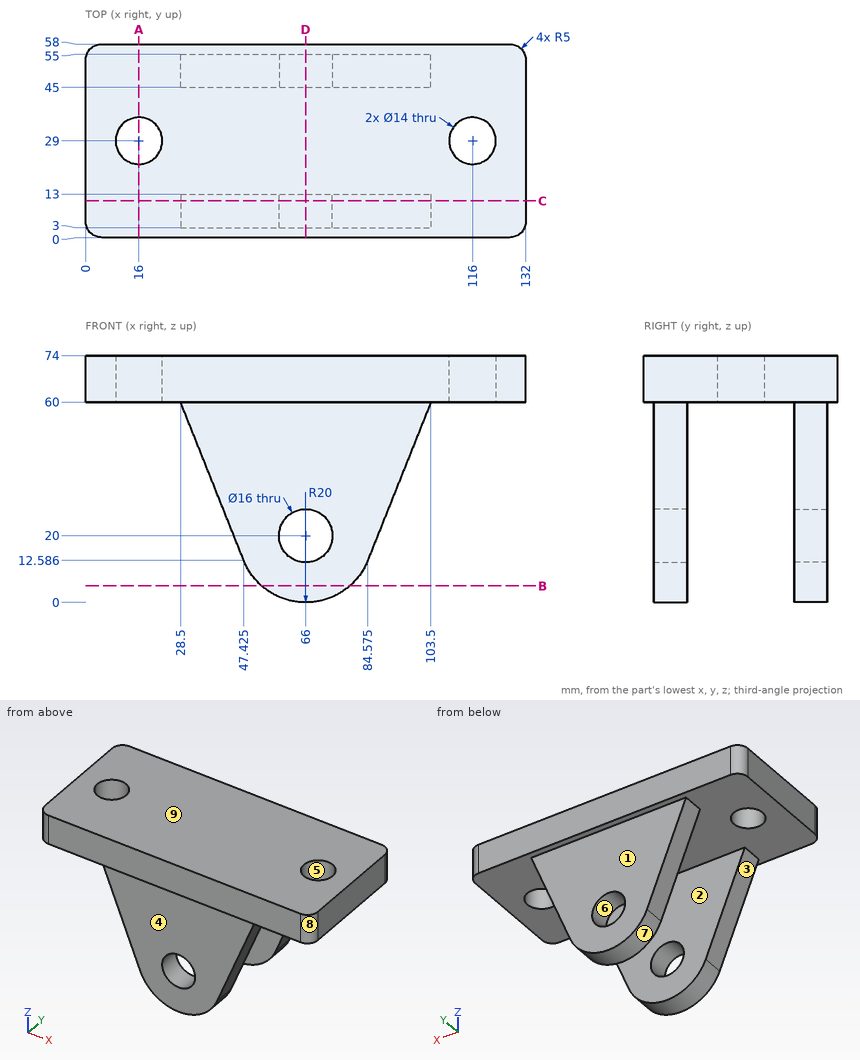
The figure shows three views and two pictorial views of one solid part (mm, origin at its lowest corner). Answer the questions. A direction names the side the tool comes from. Round coordinates to 2 decimals unless told otherwise and drop trailing zeros. Write each loop counter-clockwise with the first axis right and the second up, starting at its lowest first coordinate (ties: lowest second). Pieces come first, ordered by that corner, then holes. Notation, with made-up numbers: (25, 55) -> (51, 55) arc R21 ccw to (51, 76) -> close; hole circle Ø1 at (-25, 52.25). An arc over 180 degrees is marked (long way). Write each question's results on one line, items separated by ' | '.
Q1. Which of the six approach directions +Z, -Z, +X, -X, +Y, -Y give full straight-line access (tool end or side, diameter ignored) to the marked faces 1, 2, 3, 4 and 5?
Data:
face 1: -Z, +X, -X, +Y | face 2: -Z, +X, -X | face 3: -Z, -X, +Y, -Y | face 4: -Z, +X, -X, -Y | face 5: +Z, -Z
Q2. Section B-B, the plane z = 5 is taken. Write down the section's boundary in (x, y).
Data:
outline: (52.77, 3) -> (79.23, 3) -> (79.23, 13) -> (52.77, 13) -> close; (52.77, 45) -> (79.23, 45) -> (79.23, 55) -> (52.77, 55) -> close
Q3. Determine the mould class of the marked faces 6, 7, 8 and 9 for opening direction Z: released by +Z, released by -Z, zero draft, split by the parting line, or undercut.
Data:
face 6: undercut | face 7: released by -Z | face 8: zero draft | face 9: released by +Z
Q4. Flat-ended cylindrical pins translate along their axes: P1, Ø21, axis at x = 66, z = 20, coming from the -Y side; P2, Ø5, axis at y = 11, z = 17, coming from the -X side; P3, Ø18, axis at x = 60, z = 23, coming from the +Y side. Find the tip coordinate at first contact, or state that the pin passes through.
Data:
P1: y = 3 | P2: x = 44.67 | P3: y = 55
Q5. Section A-A, the plane x = 16 is taken. Write down the section's boundary in (y, z), then the cut area to 3 significant figures.
Data:
outline: (0, 60) -> (22, 60) -> (22, 74) -> (0, 74) -> close; (36, 60) -> (58, 60) -> (58, 74) -> (36, 74) -> close | area: 616 mm^2
Q6. Section C-C, the plane y = 11 is taken. Write down the section's boundary in (x, z) (3 decimals), then the cut area to 3 significant figures.
Data:
outline: (0, 60) -> (28.5, 60) -> (47.425, 12.586) arc R20 ccw to (84.575, 12.586) -> (103.5, 60) -> (132, 60) -> (132, 74) -> (0, 74) -> close; hole circle Ø16 at (66, 20) | area: 4,640 mm^2
Q7. Section D-D, the plane x = 66 is taken. Write down the section's boundary in (y, z), then the cut area to 3 significant figures.
Data:
outline: (0, 60) -> (3, 60) -> (3, 28) -> (13, 28) -> (13, 60) -> (45, 60) -> (45, 28) -> (55, 28) -> (55, 60) -> (58, 60) -> (58, 74) -> (0, 74) -> close; (3, 0) -> (13, 0) -> (13, 12) -> (3, 12) -> close; (45, 0) -> (55, 0) -> (55, 12) -> (45, 12) -> close | area: 1,690 mm^2
Q8. Straight lines are drawn through the part: line 1 along Y through (x, z) = (90.5, 31); line 2 along Y through (x, z) = (16, 69.5); line 3 along Z through (x, y) = (78, 23.5). For each, find the intervals that lie inside material, in ascending order. Write a range as [from, to].
Data:
line 1: [3, 13], [45, 55] | line 2: [0, 22], [36, 58] | line 3: [60, 74]
